from build123d import *

# Parameters (mm, degrees)
BOSS_EXTRUDE1_DEPTH = 5
SKETCH3_R           = 1.5
CUT_EXTRUDE1_DEPTH  = 38.057387927


with BuildPart() as part:
    # Sketch1 → Boss-Extrude1 (new body)
    with BuildSketch(Plane.XY):
        with BuildLine():
            Line((-32.5, 4), (32.5, 4))
            ThreePointArc((32.5, 4), (36.5, 0), (32.5, -4))
            Line((32.5, -4), (-32.5, -4))
            ThreePointArc((-32.5, -4), (-36.5, 0), (-32.5, 4))
        make_face()
    extrude(amount=BOSS_EXTRUDE1_DEPTH)

    # Sketch3 → Cut-Extrude1 (cut, through all)
    with BuildSketch(Plane.XY.offset(5)):
        with Locations((-32.5, 0)):
            Circle(SKETCH3_R)
        with Locations((32.5, 0)):
            Circle(SKETCH3_R)
    extrude(amount=-CUT_EXTRUDE1_DEPTH, mode=Mode.SUBTRACT)


solid = part.part
Read the model definition and answer for the solid it produces. Units are mm, in the model's axes. Coordinates: 2 decimals unless noted, no trailing zeros. Loops run counter-clockwise (first coordinate to the right, second up) from the corner with the lowest first, then second, coordinate; pieces in that order, holes last. Notation, with made-up numbers: (45, -22.75) - (62, -22.75) arc R18 ccw to (62, -0.75) - close; hole circle Ø11 at (38.5, 13.5). An arc over 180 degrees is marked (long way). Answer in a Markdown table with one row per item.
Q1. Given P1, Ø2, axis at y = -2, z = 4.5, coming from the +X side; P2, Ø1, axis at y = -3, z = 1.5, coming from the +X side, each flat-ended and moving along its own axis, determine where each tip first touches the part or whether it passes through.
Here are the results:
| item | result |
|---|---|
| P1 | stops at x = 36.37 |
| P2 | stops at x = 35.62 |
Q2. Find section B-B on z = 0.85. Write down the section's boundary in (x, y), plus the area to 3 significant figures.
Here are the results:
| item | result |
|---|---|
| outline | (-32.5, -4) - (32.5, -4) arc R4 ccw to (32.5, 4) - (-32.5, 4) arc R4 ccw to start; hole circle Ø3 at (-32.5, 0); hole circle Ø3 at (32.5, 0) |
| area | 556 mm^2 |
Q3. Find section C-C on y = -2.75. Write down the section's boundary in (x, z).
Here are the results:
| item | result |
|---|---|
| outline | (-35.4, 0) - (35.4, 0) - (35.4, 5) - (-35.4, 5) - close |
Q4. The mould has two halves that part along X. Classify faces 1 (the cylindrical face through (-33.7, -0.9, 2.5)), 2 (the cylindrical face through (-36.5, -0.1, 2.5)), 3 (the flat face through (0, -4, 2)), 4 (the cylindrical face through (31, 0, 3)): pulls with the +X half, pulls with the -X half, needs draft (parallel to the pull), parting line crosses it, or undercut.
Here are the results:
| item | result |
|---|---|
| face 1 | undercut |
| face 2 | pulls with the -X half |
| face 3 | needs draft |
| face 4 | undercut |
Q5. Straight lines are drawn through the part: line 1 along Y through (x, z) = (-32.5, 3.45); line 2 along X through (y, z) = (0.75, 2.9); line 3 along X through (y, z) = (-1.25, 3.6). For each, find the intervals that lie inside material, in ascending order. Write a range as [from, to].
Here are the results:
| item | result |
|---|---|
| line 1 | y = [-4, -1.5], [1.5, 4] |
| line 2 | x = [-36.43, -33.8], [-31.2, 31.2], [33.8, 36.43] |
| line 3 | x = [-36.3, -33.33], [-31.67, 31.67], [33.33, 36.3] |
Q6. Find section A-A on y = 0. Write down the section's boundary in (x, z), plus the area to 3 significant figures.
Here are the results:
| item | result |
|---|---|
| outline | (-36.5, 0) - (-34, 0) - (-34, 5) - (-36.5, 5) - close; (-31, 0) - (31, 0) - (31, 5) - (-31, 5) - close; (34, 0) - (36.5, 0) - (36.5, 5) - (34, 5) - close |
| area | 335 mm^2 |
